Work out the finished part from the listing and answer in its coordinate system (mm). A direction names the side the tool comes from. Coordinates: 2 decimals unless noted, no trailing zeros. Write each loop counter-clockwise with the first axis right and the second up, starting at its lowest first coordinate (ties: lowest second). Pieces come first, ordered by that corner, then holes. Notation, with made-up numbers: (-7, 83.5) - (-3, 83.5) arc R11 cw to (-3, 87.5) - close; hole circle Ø2 at (26.5, 71). An arc over 180 degrees is marked (long way). Use a Markdown table: item, result. Add a question column.
(1) The part is cut by section A-A, the plane z = -16.5. Give the vertices of the cut face in (x, y).
(2) Find the intervals of material crossed by line 1 (X direction, y = 13.25, z = -16); line 2 (Y direction, x = 49.5, z = -11); line 3 (Z direction, x = 14, y = 2.5), in increasing order. Write a range as from..to.
(3) The part is cut by section D-D, the plane z = -89. Give the vertices of the cut face in (x, y), then the cut area to 3 significant figures.
(4) The part is cut by section B-B, the plane x = 15. Give the vertices of the cut face in (y, z).
(5) For a pull along Z with two mould halves and no side action, classify faces 1 (the face through (109.1, 0.76, -0.86)), 2 (the face through (54, 0, -73)), 3 (the face through (93.017, 8.895, -16.24)) as released by +Z, released by -Z, zero draft, split by the parting line, or undercut.
(6) A tool of negligible diameter and unlimited length cuts with its end or side. For faces 4 (the face through (109.14, 0.76, -142.1)), 5 (the face through (14.912, 8.895, -124.502)), from which of +Z, -Z, +X, -X, +Y, -Y can it reach the whole face along a straight path? Write none if from no direction.
(7) The part is cut by section C-C, the plane y = 14.5. Give the vertices of the cut face in (x, z), then the cut area to 3 significant figures.
(8) Given pin 1 Ø1 at (y, z) = (3.5, -34.5) entering from -X; pin 2 Ø8 at (x, z) = (34, -61) entering from +Y, each flat-ended and moving along its own axis, determine where each tip first touches the part or whether it passes through.
from build123d import *

# Parameters (mm, degrees)
SKETCH_1_W      = 110
SKETCH_1_H      = 143
EXTRUDE_1_DEPTH = 1.5
FILLET_1_R      = 3
SKETCH_2_R      = 2
EXTRUDE_2_DEPTH = 15


with BuildPart() as part:
    # 草图1 → 凸台-拉伸1 (new body)
    with BuildSketch(Plane(origin=(0, 0, 0), x_dir=(1, 0, 0), z_dir=(0, 1, 0))):
        with Locations((55, 71.5)):
            Rectangle(SKETCH_1_W, SKETCH_1_H)
    extrude(amount=EXTRUDE_1_DEPTH)

    # 圆角1
    fillet_1_edges = [part.edges().sort_by_distance(p)[0] for p in [
        (0, 0.75, -143),
        (110, 0.75, -143),
        (110, 0.75, 0),
        (0, 0.75, 0),
    ]]
    fillet(fillet_1_edges, radius=FILLET_1_R)

    # 草图2 → 凸台-拉伸2 (add)
    with BuildSketch(Plane(origin=(0, 1.5, 0), x_dir=(1, 0, 0), z_dir=(0, 1, 0))):
        with Locations(Location((15, 126.5, 0), (0, 0, 90))):
            Circle(SKETCH_2_R)
        with Locations(Location((95, 16.5, 0), (0, 0, 90))):
            Circle(SKETCH_2_R)
        with Locations(Location((15, 16.5, 0), (0, 0, 90))):
            Circle(SKETCH_2_R)
        with Locations(Location((95, 126.5, 0), (0, 0, 90))):
            Circle(SKETCH_2_R)
    extrude(amount=EXTRUDE_2_DEPTH)


solid = part.part
Model answer:
| question | item | result |
|---|---|---|
| 1 | outline | (0, 0) - (110, 0) - (110, 1.5) - (97, 1.5) - (97, 16.5) - (93, 16.5) - (93, 1.5) - (17, 1.5) - (17, 16.5) - (13, 16.5) - (13, 1.5) - (0, 1.5) - close |
| 2 | line 1 | 13.06..16.94, 93.06..96.94 |
| 2 | line 2 | 0..1.5 |
| 2 | line 3 | -128.23..-124.77, -18.23..-14.77 |
| 3 | outline | (0, 0) - (110, 0) - (110, 1.5) - (0, 1.5) - close |
| 3 | area | 165 mm^2 |
| 4 | outline | (0, -143) - (1.5, -143) - (1.5, -128.5) - (16.5, -128.5) - (16.5, -124.5) - (1.5, -124.5) - (1.5, -18.5) - (16.5, -18.5) - (16.5, -14.5) - (1.5, -14.5) - (1.5, 0) - (0, 0) - close |
| 5 | face 1 | released by +Z |
| 5 | face 2 | zero draft |
| 5 | face 3 | undercut |
| 6 | face 4 | -Z, +X, +Y, -Y |
| 6 | face 5 | +Y |
| 7 | outline | circle Ø4 at (15, -126.5); circle Ø4 at (15, -16.5); circle Ø4 at (95, -126.5); circle Ø4 at (95, -16.5) |
| 7 | area | 50.3 mm^2 |
| 8 | pin 1 | through |
| 8 | pin 2 | y = 1.5 |
